Geometry: see drawing. Coordinates: mm, zero at the bounding-box minimum. A direction names the side the tool comes from. Round coordinates to 2 decimals unless told otherwise and drop trailing zeros. Order: outer loops, then holes, each group sorted by start corner. A loop starts at its lowest first (then second) coordinate and runs counter-clockwise, first axis right, second up. Notation, with made-up numbers: (31.25, 16) -> (50.25, 16) arc R23 cw to (50.25, 31) -> close; hole circle Ø6 at (38.25, -27.75). An arc over 180 degrees is marked (long way). One line per item, written item: value. Start each with the question number.
1) Section C-C (z = 3.25). Return the cut outline in (x, y), and give its area (3 significant figures).
2) Section A-A (y = 13.9). Return the cut outline in (x, z).
3) Mould query, pull axis X, two halves, no side actions, for the marked faces 3, 4 and 5. Classes: pulls with the +X half, pulls with the -X half, needs draft (parallel to the pull), parting line crosses it, or undercut.
4) Reachability of the marked faces 1 and 2 from +Z, -Z, +X, -X, +Y, -Y: full face, straight path, thin tool, end or side. Return the list, or none.
5) Section B-B (x = 13.9). Return the cut outline in (y, z), and give its area (3 significant figures).
6) Ray query, L1, parallel to Y at x = 13.9, z = 1.7; L2, parallel to X at y = 12, z = 4.5; L3, parallel to Y at x = 11.25, z = 5.5. Return the intervals inside material, ascending.
7) Section D-D (z = 13.5). Return the cut outline in (x, y), and give its area (3 significant figures).
8) Pin query (flat end, axial travel): P1, Ø1.5, axis at x = 11, z = 11, coming from the -Y side; P2, Ø5, axis at x = 16, z = 21, coming from the +Y side; P3, Ø4, axis at x = 12.5, y = 13.5, coming from the -Z side. Return the tip coordinate at first contact, or that it passes through.
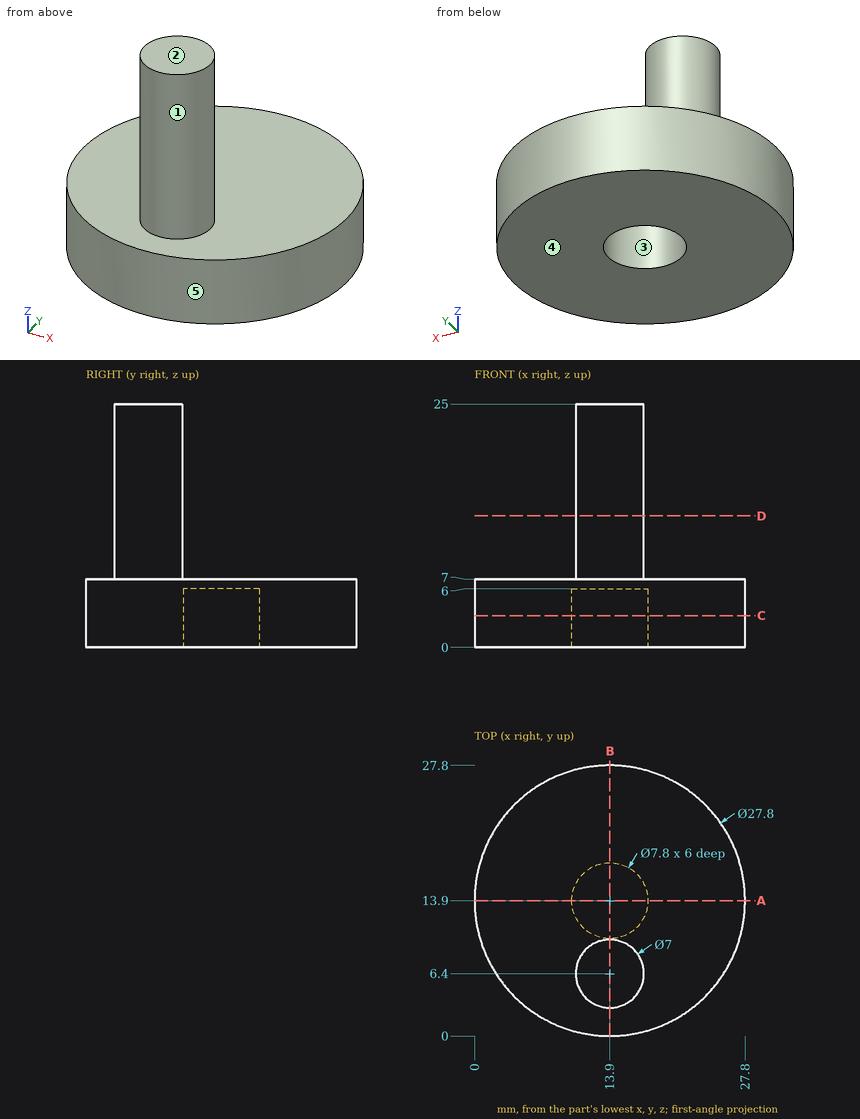
Findings:
1. outline: circle Ø27.8 at (13.9, 13.9); hole circle Ø7.8 at (13.9, 13.9)
1. area: 559 mm2
2. outline: (0, 0) -> (10, 0) -> (10, 6) -> (17.8, 6) -> (17.8, 0) -> (27.8, 0) -> (27.8, 7) -> (0, 7) -> close
3. face 3: undercut
3. face 4: needs draft
3. face 5: parting line crosses it
4. face 1: +Z
4. face 2: +Z, +X, -X, +Y, -Y
5. outline: (0, 0) -> (10, 0) -> (10, 6) -> (17.8, 6) -> (17.8, 0) -> (27.8, 0) -> (27.8, 7) -> (9.9, 7) -> (9.9, 25) -> (2.9, 25) -> (2.9, 7) -> (0, 7) -> close
5. area: 274 mm2
6. L1: 0 to 10, 17.8 to 27.8
6. L2: 0.13 to 10.49, 17.31 to 27.67
6. L3: 0.25 to 11.04, 16.76 to 27.55
7. outline: circle Ø7 at (13.9, 6.4)
7. area: 38.5 mm2
8. P1: y = 3.64
8. P2: y = 9.9
8. P3: z = 6
